from build123d import *

# Parameters (mm, degrees)
SKETCH_1_W          = 375
SKETCH_1_H          = 14
SKETCH_1_R          = 2.75
EXTRUDE_1_DEPTH     = 1.5
SKETCH_2_R          = 4
CUT_EXTRUDE_1_DEPTH = 3


with BuildPart() as part:
    # 草图1 → 凸台-拉伸1 (new, symmetric)
    with BuildSketch(Plane.XY):
        Rectangle(SKETCH_1_W, SKETCH_1_H)
        with Locations((-152.5, 0)):
            Circle(SKETCH_1_R, mode=Mode.SUBTRACT)
        with Locations((-107.5, 0)):
            Circle(SKETCH_1_R, mode=Mode.SUBTRACT)
        with Locations((-62.5, 0)):
            Circle(SKETCH_1_R, mode=Mode.SUBTRACT)
    extrude(amount=EXTRUDE_1_DEPTH, both=True)

    # 草图2 → 切除-拉伸1 (cut)
    with BuildSketch(Plane.XY.offset(1.5)):
        with Locations((156.5, 0)):
            Circle(SKETCH_2_R)
    extrude(amount=-CUT_EXTRUDE_1_DEPTH, mode=Mode.SUBTRACT)


solid = part.part
The listing builds one solid part. Answer for the finished solid, in the listing's coordinates (mm). Give positions to 0.01 mm unless a question says otherwise; leave off trailing zeros. Order: outer loops, then holes, each group sorted by start corner. A loop starts at its lowest first (then second) coordinate and runs counter-clockwise, first axis right, second up. Notation, with made-up numbers: (66.5, -13.5) -> (102.5, -13.5) arc R27 ccw to (102.5, 21.5) -> close; hole circle Ø5 at (41, 35). An arc over 180 degrees is marked (long way). Put each result on its own line as item: value.
Item 1: A cutting plane is placed at B-B on y = 0. Give the vertices of the cut face in (x, z).
Established:
outline: (-187.5, -1.5) -> (-155.25, -1.5) -> (-155.25, 1.5) -> (-187.5, 1.5) -> close; (-149.75, -1.5) -> (-110.25, -1.5) -> (-110.25, 1.5) -> (-149.75, 1.5) -> close; (-104.75, -1.5) -> (-65.25, -1.5) -> (-65.25, 1.5) -> (-104.75, 1.5) -> close; (-59.75, -1.5) -> (152.5, -1.5) -> (152.5, 1.5) -> (-59.75, 1.5) -> close; (160.5, -1.5) -> (187.5, -1.5) -> (187.5, 1.5) -> (160.5, 1.5) -> close
Item 2: A cutting plane is placed at A-A on x = 156.5. Give the vertices of the cut face in (y, z).
Established:
outline: (-7, -1.5) -> (-4, -1.5) -> (-4, 1.5) -> (-7, 1.5) -> close; (4, -1.5) -> (7, -1.5) -> (7, 1.5) -> (4, 1.5) -> close
Item 3: Straight lines are drawn through the part: line 1 (X direction, y = 0.5, z = -0.25); line 2 (Y direction, x = 156.5, z = 0.4); line 3 (Y direction, x = -152.5, z = -0.2). For each, find the intervals that lie inside material, in ascending order.
Established:
line 1: x = -187.5 to -155.2, -149.8 to -110.2, -104.8 to -65.2, -59.8 to 152.53, 160.47 to 187.5
line 2: y = -7 to -4, 4 to 7
line 3: y = -7 to -2.75, 2.75 to 7
Item 4: For a pull along X with two mould halves and no side action, classify faces 1 (the face through (160.315, 1.201, 0.021)), 2 (the face through (-3, 0, 1.5)) as released by +X, released by -X, zero draft, split by the parting line, or undercut.
Established:
face 1: undercut
face 2: zero draft
Item 5: A cutting plane is placed at C-C on z = -0.95. Give the vertices of the cut face in (x, y).
Established:
outline: (-187.5, -7) -> (187.5, -7) -> (187.5, 7) -> (-187.5, 7) -> close; hole circle Ø5.5 at (-152.5, 0); hole circle Ø5.5 at (-107.5, 0); hole circle Ø5.5 at (-62.5, 0); hole circle Ø8 at (156.5, 0)
